from build123d import *

# Parameters (mm, degrees)
SKETCH6_W                  = 50
SKETCH6_H                  = 76
BOSS_EXTRUDE6_DEPTH        = 12
M6_TAPPED_HOLE2_D          = 5
M6_TAPPED_HOLE2_DEPTH      = 15
M6_TAPPED_HOLE2_TIP        = 1.502151548
M5_TAPPED_HOLE3_AT_2_COUNT = 2
M5_TAPPED_HOLE3_AT_2_PITCH = 20
M5_TAPPED_HOLE2_D          = 4.2
M5_TAPPED_HOLE2_DEPTH      = 12.4
M5_TAPPED_HOLE2_TIP        = 1.2618073
CHAMFER1_SIZE              = 1


with BuildPart() as part:
    # Sketch6 → Boss-Extrude6 (new body)
    with BuildSketch(Plane(origin=(0, 0, 0), x_dir=(0, 0, -1), z_dir=(1, 0, 0))):
        with Locations((25, 0)):
            Rectangle(SKETCH6_W, SKETCH6_H)
    extrude(amount=-BOSS_EXTRUDE6_DEPTH)

    # M6 Tapped Hole2
    with Locations(Plane(origin=(0, 0, 0), x_dir=(0, 0, -1), z_dir=(1, 0, 0))):
        with Locations((21, -30), (21, 30)):
            Hole(M6_TAPPED_HOLE2_D / 2, depth=M6_TAPPED_HOLE2_DEPTH)
            with Locations((0, 0, -(M6_TAPPED_HOLE2_DEPTH + M6_TAPPED_HOLE2_TIP / 2))):  # 118° drill point
                Cone(0, M6_TAPPED_HOLE2_D / 2, M6_TAPPED_HOLE2_TIP, mode=Mode.SUBTRACT)

    # Sketch19 → M5 Tapped Hole3 (revolve, cut)
    with BuildSketch(Plane(origin=(-6, -38, -10), x_dir=(0, 0, -1), z_dir=(1, 0, 0))):
        Polygon((0, 0), (0, 18.6618073), (2.1, 17.4), (2.1, 0), align=None)
    m5_tapped_hole3 = revolve(axis=Axis((-6, -44.35, -10), (0, 1, 0)), mode=Mode.SUBTRACT)

    # M5 Tapped Hole3 at 2: M5 Tapped Hole3 ×2
    with Locations(*[(0, 0, -i * M5_TAPPED_HOLE3_AT_2_PITCH) for i in range(1, M5_TAPPED_HOLE3_AT_2_COUNT)]):
        add(m5_tapped_hole3, mode=Mode.SUBTRACT)

    # Mirror1: M5 Tapped Hole3 across plane
    add(m5_tapped_hole3.mirror(Plane.ZX), mode=Mode.SUBTRACT)

    # Mirror1 copy 1 sketch → Mirror1 copy 1 (revolve, cut)
    with BuildSketch(Plane(origin=(-6, 38, -30), x_dir=(0, 0, -1), z_dir=(1, 0, 0))):
        Polygon((0, 0), (0, -18.6618073), (2.1, -17.4), (2.1, 0), align=None)
    revolve(axis=Axis((-6, 44.35, -30), (0, 1, 0)), mode=Mode.SUBTRACT)

    # M5 Tapped Hole2
    with Locations(Plane.XY):
        with Locations((-6, 15), (-6, -15)):
            Hole(M5_TAPPED_HOLE2_D / 2, depth=M5_TAPPED_HOLE2_DEPTH)
            with Locations((0, 0, -(M5_TAPPED_HOLE2_DEPTH + M5_TAPPED_HOLE2_TIP / 2))):  # 118° drill point
                Cone(0, M5_TAPPED_HOLE2_D / 2, M5_TAPPED_HOLE2_TIP, mode=Mode.SUBTRACT)

    # Chamfer1
    chamfer1_edges = [part.edges().sort_by_distance(p)[0] for p in [
        (-6, 38, 0),
        (-6, 38, -50),
        (-6, -38, -50),
        (-6, -38, 0),
    ]]
    chamfer(chamfer1_edges, length=CHAMFER1_SIZE)


solid = part.part
Design review of the part built by this model. Coordinates are the model's own, in mm. A direction names the side the tool comes from. Give positions to 0.01 mm unless a question says otherwise; leave off trailing zeros. Order: outer loops, then holes, each group sorted by start corner. A loop starts at its lowest first (then second) coordinate and runs counter-clockwise, first axis right, second up. Notation, with made-up numbers: (-14, 81) - (38, 81) arc R36 ccw to (38, 118) - close; hole circle Ø3 at (82, 65.25). An arc over 180 degrees is marked (long way). Use CSV: the item, a comma, the result in double quotes. Start each with the question number.
Q1. Take a section at C-C (y = -23). State the section outline as (x, z) points.
Q2. Take a section at B-B (z = -21). State the section outline as (x, y) points, and give its area (3 significant figures).
Q3. Draft analysis for pull direction Y (two halves, no side actions). For faces 4 (the face through (-6.08, -28.31, -22.84)), 5 (the face through (-6, -1, -50)), 6 (the face through (-6.08, 31.69, -22.84)), 7 (the face through (-6.25, 19.56, -9.73)), state which applies: pulls with the +Y half, pulls with the -Y half, needs draft (parallel to the pull), parting line crosses it, or undercut.
Q4. Take a section at D-D (z = -6.5). State the section outline as (x, y) points, and give its area (3 significant figures).
Q5. Machinability: for faces 1 (the face through (-6.09, -29.42, -27.9)), 2 (the face through (-5.727, -12.918, -6.287)), 3 (the face through (-6.09, 29.42, -7.9)), which of the approach directions +Z, -Z, +X, -X, +Y, -Y give a long, thin tool a straight path to every point of the face, cutting with its end or side? Answer none if there is none.
Q6. For P1, Ø4, axis at x = -6, z = -10, coming from the +Y side; P2, Ø3.5, axis at x = -6, z = -10, coming from the -Y side, all flat-tipped, find the tip position at first contact; note any pin that passes through.
Q7. Take a section at A-A (y = 30). State the section outline as (x, z) points, and give its area (3 significant figures).
Q8. For line 1 (Y direction, x = -5.5, z = -21); line 2 (Z direction, x = -6, y = -27); line 3 (X direction, y = -27.5, z = -30), list the stretches that pass through material, from the lowest coordinate up.
Calculated:
1,outline,"(-12, -50) - (0, -50) - (0, 0) - (-12, 0) - close; hole circle Ø4.2 at (-6, -30); hole circle Ø4.2 at (-6, -10)"
2,outline,"(-12, -38) - (0, -38) - (0, -32.5) - (-12, -32.5) - close; (-12, -27.5) - (0, -27.5) - (0, 27.5) - (-12, 27.5) - close; (-12, 32.5) - (0, 32.5) - (0, 38) - (-12, 38) - close"
2,area,"792 mm²"
3,face 4,"undercut"
3,face 5,"needs draft"
3,face 6,"undercut"
3,face 7,"pulls with the +Y half"
4,outline,"(-12, -38) - (0, -38) - (0, 38) - (-12, 38) - close; hole circle Ø4.2 at (-6, -15); hole circle Ø4.2 at (-6, 15)"
4,area,"884 mm²"
5,face 1,"-Y"
5,face 2,"+Z"
5,face 3,"+Y"
6,P1,"stops at y = 20.54"
6,P2,"stops at y = -20.39"
7,outline,"(-12, -50) - (0, -50) - (0, -23.5) - (-12, -23.5) - close; (-12, -18.5) - (0, -18.5) - (0, 0) - (-12, 0) - close; hole circle Ø4.2 at (-6, -30); hole circle Ø4.2 at (-6, -10)"
7,area,"512 mm²"
8,line 1,"y = -38 to -32.5, -27.5 to 27.5, 32.5 to 38"
8,line 2,"z = -50 to -32.1, -27.9 to -12.1, -7.9 to 0"
8,line 3,"x = -12 to -8.1, -3.9 to 0"
